```python
from build123d import *

# Parameters (mm, degrees)
BRACKET_BODY_DEPTH        = 40
BASE_NOTCH_SKETCH_W       = 30
BASE_NOTCH_SKETCH_H       = 7
BASE_NOTCH_CUT_DEPTH      = 63.801273872
CYLINDRICAL_BOSS_DEPTH    = 20
UPRIGHT_OPENING_SKETCH_W  = 8
UPRIGHT_OPENING_SKETCH_H  = 5
UPRIGHT_OPENING_CUT_DEPTH = 20
ARCHED_RELIEF_CUT_DEPTH   = 59.685603004
SUPPORT_RIB_45DEG_REACH   = 54.383
SUPPORT_RIB_SKETCH_WALL_W = 126.565396702
SUPPORT_RIB_SKETCH_WALL_H = 5


with BuildPart() as part:
    # Bracket Profile Sketch → Bracket Body (new body)
    with BuildSketch(Plane.XY):
        Polygon((0, 0), (30, 0), (30, 38), (20, 38), (20, 12), (0, 12), align=None)
    extrude(amount=BRACKET_BODY_DEPTH)

    # Base Notch Sketch → Base Notch Cut (cut, through all)
    with BuildSketch(Plane.ZY):
        with Locations((20, 3.5)):
            Rectangle(BASE_NOTCH_SKETCH_W, BASE_NOTCH_SKETCH_H)
    extrude(amount=-BASE_NOTCH_CUT_DEPTH, mode=Mode.SUBTRACT)

    # Cylindrical Boss Sketch → Cylindrical Boss (add)
    with BuildSketch(Plane.ZY):
        with BuildLine():
            Line((13, 7), (13, 17))
            ThreePointArc((13, 17), (20, 24), (27, 17))
            Line((27, 17), (27, 7))
            ThreePointArc((27, 7), (20, 0), (13, 7))
        make_face()
        with BuildLine():
            Line((16, 7), (16, 17))
            ThreePointArc((16, 17), (20, 21), (24, 17))
            Line((24, 17), (24, 7))
            ThreePointArc((24, 7), (20, 3), (16, 7))
        make_face(mode=Mode.SUBTRACT)
    extrude(amount=-CYLINDRICAL_BOSS_DEPTH)

    # Upright Opening Sketch → Upright Opening Cut (cut)
    with BuildSketch(Plane.ZY):
        with Locations((20, 9.5)):
            Rectangle(UPRIGHT_OPENING_SKETCH_W, UPRIGHT_OPENING_SKETCH_H)
    extrude(amount=-UPRIGHT_OPENING_CUT_DEPTH, mode=Mode.SUBTRACT)

    # Arched Relief Sketch → Arched Relief Cut (cut, through all)
    with BuildSketch(Plane.ZY.offset(-20)):
        with BuildLine():
            Line((16, 17), (16, 7))
            Line((16, 7), (24, 7))
            Line((24, 7), (24, 17))
            ThreePointArc((24, 17), (20, 21), (16, 17))
        make_face()
    extrude(amount=-ARCHED_RELIEF_CUT_DEPTH, mode=Mode.SUBTRACT)

    # Support Rib Sketch wall → Support Rib 45deg (add, up to next)
    with BuildSketch(Plane(origin=(13, 31, 20), x_dir=(-0.707106781187, -0.707106781187, 0), z_dir=(0.707106781187, -0.707106781187, 0)), mode=Mode.PRIVATE) as support_rib_45deg_sk1:
        Rectangle(SUPPORT_RIB_SKETCH_WALL_W, SUPPORT_RIB_SKETCH_WALL_H)
    support_rib_45deg_tool1 = extrude(support_rib_45deg_sk1.sketch, amount=SUPPORT_RIB_45DEG_REACH, mode=Mode.PRIVATE) - part.part
    add(support_rib_45deg_tool1.solids().sort_by_distance((13, 31, 20))[0])


solid = part.part
```
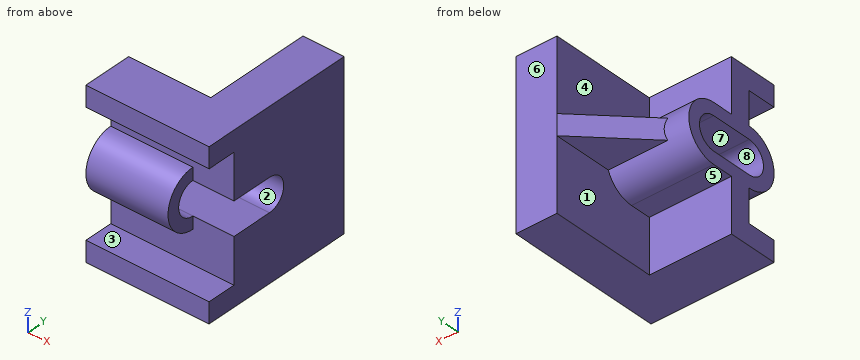
Work out the finished part from the listing and answer in its coordinate system (mm). Face numbers are marked on the shaded views. A direction names the side the tool comes from. Give positions to 0.01 mm unless a question says otherwise; leave off trailing zeros. Loops run counter-clockwise (first coordinate to the right, second up) from the corner with the lowest first, then second, coordinate; pieces in that order, holes last. Notation, with made-up numbers: M -10,2.25 L 49,2.25 A32 cw 49,39.25 Z; hole C 26,35 d2. An arc over 180 degrees is marked long. One line per item, written item: value. Start each with the question number.
1. Determine the mould class of the marked faces 5, 6, 7 and 8 for opening direction Y: released by +Y, released by -Y, zero draft, split by the parting line, or undercut.
2. Find section B-B (x = 23.75). Give the vertices of the cut face in (y, z), and give its area (3 significant figures).
3. Find the intervals of material crossed by probe 1 along Z at (x, y) = (5.75, 9); probe 2 along Z at (x, y) = (3, 16); probe 3 along X at (y, z) = (26.5, 30), in increasing order.
4. Find section D-D (x = 14.75). Give the vertices of the cut face in (y, z).
5. Which of the six approach directions +Z, -Z, +X, -X, +Y, -Y give full straight-line access (tool end or side, diameter ignored) to the marked faces 1, 2, 3 and 4?
6. Find section A-A (z = 20). Give the vertices of the cut face in (x, y), and give its area (3 significant figures).
7. Each of these flat-tipped pins is pushed along its axis until it touches: P1, Ø4.5, axis at x = 10, y = 33, coming from the -Z side; P2, Ø10.5, axis at x = 13, z = 7.5, coming from the +Y side; P3, Ø12, axis at x = 19.5, z = 8, coming from the -Y side; P4, Ø7, axis at x = 16, y = 30.5, coming from the +Z side. Where does it stop, or does it pass through?
8. Find section C-C (y = 18). Give the vertices of the cut face in (x, z).
Reported:
1. face 5: zero draft
1. face 6: released by +Y
1. face 7: undercut
1. face 8: undercut
2. outline: M 0,0 L 38,0 L 38,40 L 0,40 L 0,35 L 7,35 L 7,24 L 17,24 A4 cw 17,16 L 7,16 L 7,5 L 0,5 Z
2. area: 1,200 mm²
3. probe 1: z = 0 to 16, 24 to 40
3. probe 2: z = 13 to 16, 24 to 27
3. probe 3: x = 20 to 30
4. outline: M 0,0 L 12,0 L 12,13 L 17,13 A7 ccw 23.54,17.5 L 32.75,17.5 L 32.75,22.5 L 23.54,22.5 A7 ccw 17,27 L 12,27 L 12,40 L 0,40 L 0,35 L 7,35 L 7,27 A7 ccw 7,13 L 7,5 L 0,5 Z; hole M 7,16 L 17,16 A4 ccw 17,24 L 7,24 A4 ccw Z
5. face 1: -Z, -X, +Y
5. face 2: +X, -X
5. face 3: +X, -X, -Y
5. face 4: +Z, -X, +Y
6. outline: M 0,0 L 20,0 L 20,3 L 0,3 Z; M 0,21 L 30,21 L 30,38 L 20,38 L 6,24 L 0,24 Z
6. area: 388 mm²
7. P1: passes through
7. P2: stops at y = 12
7. P3: stops at y = 0
7. P4: stops at z = 22.5
8. outline: M 0,13.07 L 20,13.07 L 20,0 L 30,0 L 30,16.13 L 0,16.13 Z; M 0,23.87 L 30,23.87 L 30,40 L 20,40 L 20,26.93 L 0,26.93 Z
